Verification items for the finished model (mm, model axes). Round coordinates to 2 decimals unless told otherwise and drop trailing zeros. Write each loop counter-clockwise with the first axis right and the second up, starting at its lowest first coordinate (ties: lowest second). Pieces come first, ordered by that corner, then holes.
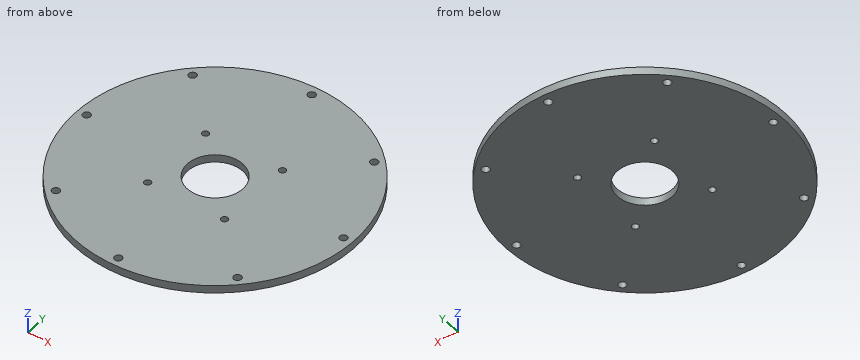
from build123d import *

# Parameters (mm, degrees)
SKETCH_1_R               = 91
SKETCH_1_R_2             = 18
EXTRUDE_1_DEPTH          = 2.5
SKETCH_2_R               = 2.5
CUT_EXTRUDE_1_DEPTH      = 5
PATTERN_CIRCULAR_1_COUNT = 8
SKETCH_3_R               = 2.2
CUT_EXTRUDE_2_DEPTH      = 10
PATTERN_CIRCULAR_2_COUNT = 4


with BuildPart() as part:
    # 草图1 → 凸台-拉伸1 (new, symmetric)
    with BuildSketch(Plane.XY):
        Circle(SKETCH_1_R)
        Circle(SKETCH_1_R_2, mode=Mode.SUBTRACT)
    extrude(amount=EXTRUDE_1_DEPTH, both=True)

    # 草图2 → 切除-拉伸1 (cut)
    with BuildSketch(Plane.XY.offset(2.5)):
        with Locations((0, 85)):
            Circle(SKETCH_2_R)
    cut_extrude_1 = extrude(amount=-CUT_EXTRUDE_1_DEPTH, mode=Mode.SUBTRACT)

    # 阵列(圆周)1: 切除-拉伸1 ×8 about axis
    pattern_circular_1_axis = Axis((0, 0, 0), (0, 0, 1))
    for i in range(1, PATTERN_CIRCULAR_1_COUNT):
        add(cut_extrude_1.rotate(pattern_circular_1_axis, i * 360 / PATTERN_CIRCULAR_1_COUNT), mode=Mode.SUBTRACT)

    # 草图3 → 切除-拉伸2 (cut)
    with BuildSketch(Plane(origin=(0, 0, -2.5), x_dir=(-1, 0, 0), z_dir=(0, 0, -1))):
        with Locations((25.455844123, 25.455844123)):
            Circle(SKETCH_3_R)
    cut_extrude_2 = extrude(amount=-CUT_EXTRUDE_2_DEPTH, mode=Mode.SUBTRACT)

    # 阵列(圆周)2: 切除-拉伸2 ×4 about axis
    pattern_circular_2_axis = Axis((0, 0, 0), (0, 0, 1))
    for i in range(1, PATTERN_CIRCULAR_2_COUNT):
        add(cut_extrude_2.rotate(pattern_circular_2_axis, i * 360 / PATTERN_CIRCULAR_2_COUNT), mode=Mode.SUBTRACT)


solid = part.part
Q1. Material ranges on line 1 along Y through (x, z) = (0, 0.9); line 2 along X through (y, z) = (23.5, 1.75); line 3 along Y through (x, z) = (15, 0.05), recorded low to high.
Recorded:
line 1: y = -91 to -87.5, -82.5 to -18, 18 to 82.5, 87.5 to 91
line 2: x = -87.91 to -26.46, -24.45 to 24.45, 26.46 to 87.91
line 3: y = -89.76 to -9.95, 9.95 to 89.76
Q2. Sectioned sample at A-A (y = 0). Enter the section's corners in (x, z).
Recorded:
outline: (-91, -2.5) - (-87.5, -2.5) - (-87.5, 2.5) - (-91, 2.5) - close; (-82.5, -2.5) - (-18, -2.5) - (-18, 2.5) - (-82.5, 2.5) - close; (18, -2.5) - (82.5, -2.5) - (82.5, 2.5) - (18, 2.5) - close; (87.5, -2.5) - (91, -2.5) - (91, 2.5) - (87.5, 2.5) - close
Q3. Sectioned sample at D-D (y = -85). Enter the section's corners in (x, z), plus the area to 3 significant figures.
Recorded:
outline: (-32.5, -2.5) - (-2.5, -2.5) - (-2.5, 2.5) - (-32.5, 2.5) - close; (2.5, -2.5) - (32.5, -2.5) - (32.5, 2.5) - (2.5, 2.5) - close
area: 300 mm2
Q4. Depth check by flat-ended pin: P1, Ø2.5, axis at x = -25.46, y = 25.46, coming from the -Z side; P2, Ø2, axis at y = -27.5, z = 0, coming from the -X side; P3, Ø2, axis at x = -34, z = 0.5, coming from the +Y side. Enter the tip coordinate at first touch or a pass-through.
Recorded:
P1: passes through
P2: stops at x = -87.06
P3: stops at y = 84.81
Q5. Sectioned sample at C-C (z = 1.4). Give the number of separate pieces and of enclosed holes in the cut face, plus the area to 3 significant figures.
Recorded:
separate pieces: 1
enclosed holes: 13
area: 24,800 mm2
